Input: part model. Units: mm. Frame: model coordinates. A direction names the side the tool comes from. Round coordinates to 2 decimals unless told otherwise and drop trailing zeros. Loops run counter-clockwise (first coordinate to the right, second up) from the corner with the lowest first, then second, coordinate; pieces in that order, holes last. Notation, with made-up numbers: (59, -23.75) - (97, -23.75) arc R22 ccw to (97, 11.25) - close; hole circle Ø6 at (88, -30.75). An arc over 180 degrees is marked (long way). Use CSV: the item, a comma, the result in double quotes. Start each with the question number.
1. Access query for faces 4 (the flat face through (2, 40, 123)), 5 (the flat face through (24, 4, 123)). Directions: +Z, -Z, +X, -X, +Y, -Y. A direction counts if a zero-diameter tool reaches every point of the face in a straight line with its end or side. Return the directions, or none.
2. Material intervals for probe 1 along Y at (x, z) = (2, 50); probe 2 along Y at (x, z) = (37.5, 194), sorted ascending. Write a range as from..to.
3. Pin query (flat end, axial travel): P1, Ø1, axis at y = 30, z = 157.5, coming from the +X side; P2, Ø12, axis at x = 16.5, z = 160.5, coming from the +Y side; P3, Ø4, axis at x = 11, y = 7.5, coming from the -Z side; P4, Ø3, axis at y = 9.5, z = 211, coming from the +X side. Return the tip coordinate at first contact, or that it passes through.
4. Pull-direction query (Y, two-part tool) for faces 1 (the cylindrical face through (5, 6, 123)), 2 (the cylindrical face through (2.028, 25.242, 205.495)), 3 (the flat face through (12.7, 3.8, 0)); classes: +Y half, -Y half, draft (parallel to the pull), parting line (faces both ways), or undercut.
5. Cut plane D-D (x = 29.5). Return loops of the section in (y, z).
6. Cut plane A-A (y = 25). Return loops of the section in (x, z), and give its area (3 significant figures).
```python
from build123d import *

# Parameters (mm, degrees)
EXTRUDE_1_DEPTH             = 250
HOLE_WIZARD_11_0_11_1_D     = 11
HOLE_WIZARD_11_0_11_1_DEPTH = 10
HOLE_WIZARD_11_0_11_1_TIP   = 3.304733405


with BuildPart() as part:
    # 草图1 → 拉伸1 (new body)
    with BuildSketch(Plane.XY):
        with BuildLine():
            Line((0, 0), (0, 40))
            Line((0, 40), (3.99, 40))
            ThreePointArc((3.99, 40), (3.997071068, 39.997071068), (4, 39.99))
            Line((4, 39.99), (4, 9))
            ThreePointArc((4, 9), (5.464466094, 5.464466094), (9, 4))
            Line((9, 4), (39.99, 4))
            ThreePointArc((39.99, 4), (39.997071068, 3.997071068), (40, 3.99))
            Line((40, 3.99), (40, 0))
            Line((40, 0), (0, 0))
        make_face()
    extrude(amount=EXTRUDE_1_DEPTH)

    # Ø11.0 (11) 直径孔1
    with Locations(Plane.ZY):
        with Locations((200, 25), (50, 25)):
            Hole(HOLE_WIZARD_11_0_11_1_D / 2, depth=HOLE_WIZARD_11_0_11_1_DEPTH)
            with Locations((0, 0, -(HOLE_WIZARD_11_0_11_1_DEPTH + HOLE_WIZARD_11_0_11_1_TIP / 2))):  # 118° drill point
                Cone(0, HOLE_WIZARD_11_0_11_1_D / 2, HOLE_WIZARD_11_0_11_1_TIP, mode=Mode.SUBTRACT)


solid = part.part
```
Established:
1,face 4,"+Z, -Z, +X, -X, +Y"
1,face 5,"+Z, -Z, +X, +Y"
2,probe 1,"y = 0..19.5, 30.5..40"
2,probe 2,"y = 0..4"
3,P1,"stops at x = 4"
3,P2,"stops at y = 4"
3,P3,"passes through"
3,P4,"stops at x = 4.1"
4,face 1,"+Y half"
4,face 2,"undercut"
4,face 3,"draft"
5,outline,"(0, 0) - (4, 0) - (4, 250) - (0, 250) - close"
6,outline,"(0, 0) - (4, 0) - (4, 44.5) - (0, 44.5) - close; (0, 55.5) - (4, 55.5) - (4, 194.5) - (0, 194.5) - close; (0, 205.5) - (4, 205.5) - (4, 250) - (0, 250) - close"
6,area,"912 mm2"
